from build123d import *

# Parameters (mm, degrees)
SKETCH_1_R          = 9.646875
EXTRUDE_483_DEPTH   = 20.2
SKETCH_2_OUTSIDE_W  = 163.884
SKETCH_2_OUTSIDE_H  = 158.886
SKETCH_2_OUTSIDE_R  = 16.151373781
CUT_EXTRUDE_1_DEPTH = 32.886194113
CUT_EXTRUDE_1_DRAFT = -60
SKETCH_3_OUTSIDE_W  = 163.884
SKETCH_3_OUTSIDE_H  = 158.886
SKETCH_3_OUTSIDE_R  = 16.151373781
CUT_EXTRUDE_2_DEPTH = 32.886194113
CUT_EXTRUDE_2_DRAFT = -60
CHAMFER_1_SIZE      = 0.505


with BuildPart() as part:
    # 草图1 → Extrude 483 (new body)
    with BuildSketch(Plane.XY):
        Polygon((9.325, 16.151373781), (-9.325, 16.151373781), (-18.65, 0), (-9.325, -16.151373781), (9.325, -16.151373781), (18.65, 0), align=None)
        Circle(SKETCH_1_R, mode=Mode.SUBTRACT)
    extrude(amount=EXTRUDE_483_DEPTH)


with BuildPart() as cut_extrude_1_tool:
    # 草图2 outside → 切除-拉伸1 (with draft: the straight prism first)
    with BuildSketch(Plane(origin=(0, 0, 0), x_dir=(-1, 0, 0), z_dir=(0, 0, -1))):
        Rectangle(SKETCH_2_OUTSIDE_W, SKETCH_2_OUTSIDE_H)
        Circle(SKETCH_2_OUTSIDE_R, mode=Mode.SUBTRACT)
    extrude(amount=-CUT_EXTRUDE_1_DEPTH)
    # 切除-拉伸1: the draft: its side faces are tilted about the plane it starts from
    cut_extrude_1_sides = [cut_extrude_1_tool.faces().sort_by_distance(p)[0] for p in [
        (0, -79.443, 16.443097056),
        (-81.942, 0, 16.443097056),
        (0, 79.443, 16.443097056),
        (81.942, 0, 16.443097056),
        (16.151373781, 0, 16.443097056),
    ]]
    draft(cut_extrude_1_sides, Plane(origin=(0, 0, 0), x_dir=(-1, 0, 0), z_dir=(0, 0, -1)), CUT_EXTRUDE_1_DRAFT)


with BuildPart() as part_1:
    add(part.part)

    # 切除-拉伸1: cut by cut_extrude_1_tool
    add(cut_extrude_1_tool.part, mode=Mode.SUBTRACT)


with BuildPart() as cut_extrude_2_tool:
    # 草图3 outside → 切除-拉伸2 (with draft: the straight prism first)
    with BuildSketch(Plane.XY.offset(20.2)):
        Rectangle(SKETCH_3_OUTSIDE_W, SKETCH_3_OUTSIDE_H)
        Circle(SKETCH_3_OUTSIDE_R, mode=Mode.SUBTRACT)
    extrude(amount=-CUT_EXTRUDE_2_DEPTH)
    # 切除-拉伸2: the draft: its side faces are tilted about the plane it starts from
    cut_extrude_2_sides = [cut_extrude_2_tool.faces().sort_by_distance(p)[0] for p in [
        (0, -79.443, 3.756902944),
        (81.942, 0, 3.756902944),
        (0, 79.443, 3.756902944),
        (-81.942, 0, 3.756902944),
        (-16.151373781, 0, 3.756902944),
    ]]
    draft(cut_extrude_2_sides, Plane.XY.offset(20.2), CUT_EXTRUDE_2_DRAFT)


with BuildPart() as part_2:
    add(part_1.part)

    # 切除-拉伸2: cut by cut_extrude_2_tool
    add(cut_extrude_2_tool.part, mode=Mode.SUBTRACT)

    # 倒角1
    chamfer_1_edges = [part_2.edges().sort_by_distance(p)[0] for p in [
        (-9.646875, 0, 0),
        (-9.646875, 0, 20.2),
    ]]
    chamfer(chamfer_1_edges, length=CHAMFER_1_SIZE)


solid = part_2.part
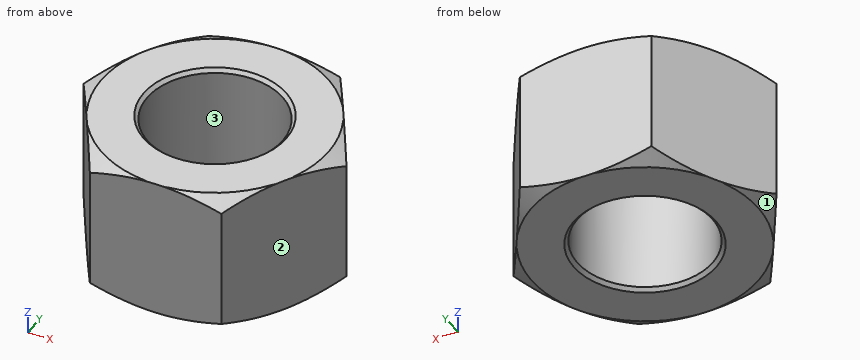
The model under review builds one solid part; all positions refer to its coordinate system, in mm. Face numbers are marked on the shaded views. Coordinates: 2 decimals unless noted, no trailing zeros. Order: outer loops, then holes, each group sorted by start corner. A loop starts at its lowest first (then second) coordinate and runs counter-clockwise, first axis right, second up. Notation, with made-up numbers: (77.5, -2) -> (118.5, -2) arc R18 ccw to (118.5, 32) -> close; hole circle Ø8 at (62.5, 87.25). An arc over 180 degrees is marked (long way). Answer in a Markdown table with one row per item.
(1) Consider section A-A (z = 7.25). Write out the cut boundary in (x, y) (3 decimals).
Answers:
| item | result |
|---|---|
| outline | (-18.65, 0) -> (-9.325, -16.151) -> (9.325, -16.151) -> (18.65, 0) -> (9.325, 16.151) -> (-9.325, 16.151) -> close; hole circle Ø19.294 at (0, 0) |
(2) Insertion check: pin 1 (6 mm diameter, centred on y = 8, z = 8, fed in from -X); pin 2 (3 mm diameter, centred on y = -7, z = 10, fed in from +X); pin 3 (5 mm diameter, centred on y = -5, z = 10.5, fed in from -X); pin 4 (6 mm diameter, centred on x = -9.5, y = 13, fed in from -Z). Each pin has a flat end and moves straight along its axis. Give the tip position at first contact, or say it passes through.
Answers:
| item | result |
|---|---|
| pin 1 | x = -15.76 |
| pin 2 | x = 15.47 |
| pin 3 | x = -17.21 |
| pin 4 | z = 0 |
(3) The part is to be moulded in two halves that separate along Y. For the marked faces 1, 2 and 3, say which applies: +Y half, -Y half, draft (parallel to the pull), parting line (faces both ways), or undercut.
Answers:
| item | result |
|---|---|
| face 1 | parting line |
| face 2 | -Y half |
| face 3 | undercut |
(4) Wall thickness on line 1 along Y through (x, z) = (3, 12.5); line 2 along Y through (x, z) = (-3.5, 14); line 3 along X through (y, z) = (6, 16.25): over which ranges is each line inside the solid? List them lowest first.
Answers:
| item | result |
|---|---|
| line 1 | -16.15 to -9.17, 9.17 to 16.15 |
| line 2 | -16.15 to -8.99, 8.99 to 16.15 |
| line 3 | -15.19 to -7.55, 7.55 to 15.19 |
